```python
from build123d import *

# Parameters (mm, degrees)
SKETCH1_R           = 4
SKETCH1_R_2         = 3.3235
BOSS_EXTRUDE1_DEPTH = 19
CUT_EXTRUDE1_REACH  = 120.448
SKETCH2_W           = 20
SKETCH2_H           = 8
SKETCH3_R           = 2.4585
CUT_EXTRUDE2_DEPTH  = 15


with BuildPart() as part:
    # Sketch1 → Boss-Extrude1 (new body)
    with BuildSketch(Plane.XY):
        Polygon((0, 0), (56, 0), (71, -5), (71, -16), (113, -16), (113, 14), (93, 14), (60, 25), (0, 25), align=None)
        with Locations((10, 12.5)):
            Circle(SKETCH1_R, mode=Mode.SUBTRACT)
        with Locations((25, 12.5)):
            Circle(SKETCH1_R_2, mode=Mode.SUBTRACT)
        with Locations((40, 12.5)):
            Circle(SKETCH1_R, mode=Mode.SUBTRACT)
    extrude(amount=BOSS_EXTRUDE1_DEPTH)

    # Sketch2 → Cut-Extrude1 (cut, up to next)
    with BuildSketch(Plane(origin=(0, 14, 0), x_dir=(1, 0, 0), z_dir=(0, 1, 0)), mode=Mode.PRIVATE) as cut_extrude1_sk1:
        with Locations((103, -9.5)):
            Rectangle(SKETCH2_W, SKETCH2_H)
    cut_extrude1_tool1 = extrude(cut_extrude1_sk1.sketch, amount=-CUT_EXTRUDE1_REACH, mode=Mode.PRIVATE) & part.part
    add(cut_extrude1_tool1.solids().sort_by_distance((103, 14, 9.5))[0], mode=Mode.SUBTRACT)

    # Sketch3 → Cut-Extrude2 (cut)
    with BuildSketch(Plane(origin=(0, -16, 0), x_dir=(-1, 0, 0), z_dir=(0, -1, 0))):
        with Locations(Location((-79, -9.5, 0), (0, 0, 180))):
            Circle(SKETCH3_R)
    extrude(amount=-CUT_EXTRUDE2_DEPTH, mode=Mode.SUBTRACT)


solid = part.part
```
Design review of the part built by this model. Coordinates are the model's own, in mm. A direction names the side the tool comes from. Coordinates: 2 decimals unless noted, no trailing zeros. Order: outer loops, then holes, each group sorted by start corner. A loop starts at its lowest first (then second) coordinate and runs counter-clockwise, first axis right, second up. Notation, with made-up numbers: M -8.5,56.25 L 12.5,56.25 A28 cw 12.5,93.25 Z; hole C 47,72 d11. An arc over 180 degrees is marked long. Answer as a JSON object with one key per item and string values. Group by question number.
1) Add section C-C, the plane y = 2.5. Write out the cut boundary in (x, z), then the cut area to 3 significant figures.
2) Add section B-B, the plane z = 2. Write out the cut boundary in (x, y), then the cut area to 3 significant figures.
3) Wall thickness on L1, parallel to Y at x = 25, z = 4.5; L2, parallel to Z at x = 99.5, y = -10.5; L3, parallel to Z at x = 79, y = -9: over which ranges is each line inside the solid? List them lowest first.
4) Add section D-D, the plane y = 12.5. Write out the cut boundary in (x, z), then the cut area to 3 significant figures.
5) For pin 1 (1.6 mm diameter, centred on x = 105.5, z = 2.5, fed in from +Y); pin 2 (4 mm diameter, centred on x = 79, z = 9.5, fed in from +Y); pin 3 (3.5 mm diameter, centred on y = -13, z = 5.5, fed in from -X), all flat-tipped, find the tip position at first contact; note any pin that passes through.
6) Mouldability with a two-part tool opening along X and no side actions: class faces 1 (the flat face through (0, 13, 9)), 2 (the flat face through (76.731, 19.423, 9.367)), 3 (the cylindrical face through (37.05, 15.2, 9.37)) as pulls with the +X half, pulls with the -X half, needs draft (parallel to the pull), parting line crosses it, or undercut.
7) Tool access review of faces 4 (the flat face through (103, 14, 16)), 5 (the flat face through (103, -1, 5.5)), 6 (the flat face through (28, 0, 9)), 7 (the cylindrical face through (81.345, -8.605, 10.238)): name each direction out of +Z, -Z, +X, -X, +Y, -Y from which nothing blocks a thin tool from reaching the whole face with its end or side.
8) Add section A-A, the plane x = 25. Write out the cut boundary in (y, z), then the cut area to 3 significant figures.
Computed values:
{
 "1": {"outline": "M 0,0 L 113,0 L 113,5.5 L 93,5.5 L 93,13.5 L 113,13.5 L 113,19 L 0,19 Z", "area": "1,990 mm^2"},
 "2": {"outline": "M 0,0 L 56,0 L 71,-5 L 71,-16 L 113,-16 L 113,14 L 93,14 L 60,25 L 0,25 Z; hole C 10,12.5 d8; hole C 25,12.5 d6.65; hole C 40,12.5 d8", "area": "3,000 mm^2"},
 "3": {"L1": "y = 0 to 9.18, 15.82 to 25", "L2": "z = 0 to 5.5, 13.5 to 19", "L3": "z = 0 to 7.04, 11.96 to 19"},
 "4": {"outline": "M 0,0 L 6,0 L 6,19 L 0,19 Z; M 14,0 L 21.68,0 L 21.68,19 L 14,19 Z; M 28.32,0 L 36,0 L 36,19 L 28.32,19 Z; M 44,0 L 113,0 L 113,5.5 L 93,5.5 L 93,13.5 L 113,13.5 L 113,19 L 44,19 Z", "area": "1,560 mm^2"},
 "5": {"pin 1": "stops at y = 14", "pin 2": "stops at y = 19.33", "pin 3": "stops at x = 71"},
 "6": {"face 1": "pulls with the -X half", "face 2": "pulls with the +X half", "face 3": "undercut"},
 "7": {"face 4": "+Z, -Z, +X, +Y", "face 5": "+X, +Y, -Y", "face 6": "+Z, -Z, -X, -Y", "face 7": "-Y"},
 "8": {"outline": "M 0,0 L 9.18,0 L 9.18,19 L 0,19 Z; M 15.82,0 L 25,0 L 25,19 L 15.82,19 Z", "area": "349 mm^2"}
}
